Study the drawing (mm; zero at the part's minimum x, y, z) and answer. Round coordinates to 2 decimals unless told otherwise and drop trailing zeros. Loops run counter-clockwise (first coordinate to the right, second up) from the corner with the lowest first, then second, coordinate; pieces in that order, holes last. Notation, with made-up numbers: (43, 50) -> (86, 50) arc R26 cw to (86, 65) -> close; hole circle Ø2 at (77.5, 3.25). An arc over 180 degrees is marked (long way). Answer in a Markdown table with one row per item. Add a question column.
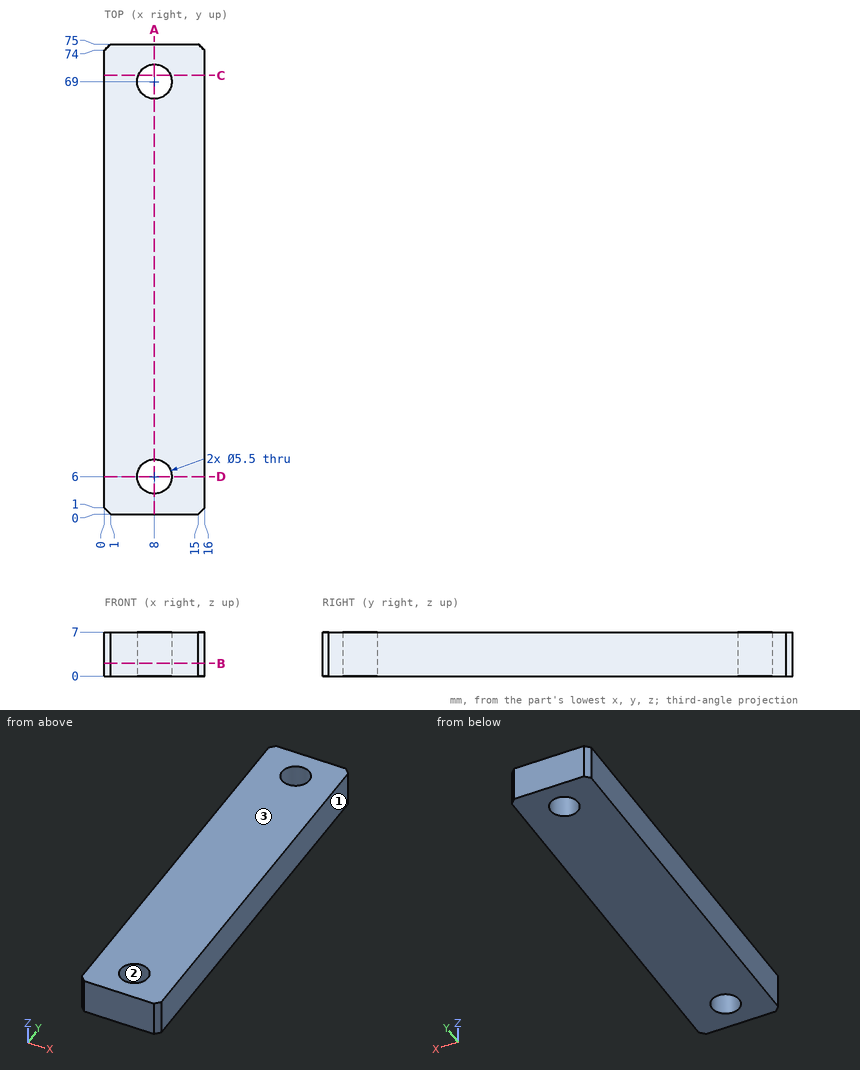
Item 1: Section D-D, the plane y = 6 is taken. Write down the section's boundary in (x, z).
Item 2: Section B-B, the plane z = 2 is taken. Write down the section's boundary in (x, y).
Item 3: Section A-A, the plane x = 8 is taken. Write down the section's boundary in (y, z).
Item 4: The mould has two halves that part along X. Classify the marked faces 1, 2 and 3: +X half, -X half, draft (parallel to the pull), parting line (faces both ways), or undercut.
Item 5: Flat-ended cylindrical pins translate along their axes: P1, Ø6.5, axis at x = 8, y = 6, coming from the +Z side; P2, Ø5, axis at x = 8, y = 69, coming from the +Z side. Find the tip coordinate at first contact, or state that the pin passes through.
Item 6: Section C-C, the plane y = 70 is taken. Write down the section's boundary in (x, z), and give its area (3 significant figures).
Item 7: Consider L1, parallel to Y at x = 8, z = 3.5; L2, parallel to Y at x = 6, z = 2.25; L3, parallel to X at y = 6.5, z = 3. Determine where each line is inside the solid, lowest interval first. Write a range as from..to.
Here are the results:
| question | item | result |
|---|---|---|
| 1 | outline | (0, 0) -> (5.25, 0) -> (5.25, 7) -> (0, 7) -> close; (10.75, 0) -> (16, 0) -> (16, 7) -> (10.75, 7) -> close |
| 2 | outline | (0, 1) -> (1, 0) -> (15, 0) -> (16, 1) -> (16, 74) -> (15, 75) -> (1, 75) -> (0, 74) -> close; hole circle Ø5.5 at (8, 6); hole circle Ø5.5 at (8, 69) |
| 3 | outline | (0, 0) -> (3.25, 0) -> (3.25, 7) -> (0, 7) -> close; (8.75, 0) -> (66.25, 0) -> (66.25, 7) -> (8.75, 7) -> close; (71.75, 0) -> (75, 0) -> (75, 7) -> (71.75, 7) -> close |
| 4 | face 1 | +X half |
| 4 | face 2 | undercut |
| 4 | face 3 | draft |
| 5 | P1 | stops at z = 7 |
| 5 | P2 | passes through |
| 6 | outline | (0, 0) -> (5.44, 0) -> (5.44, 7) -> (0, 7) -> close; (10.56, 0) -> (16, 0) -> (16, 7) -> (10.56, 7) -> close |
| 6 | area | 76.1 mm² |
| 7 | L1 | y = 0..3.25, 8.75..66.25, 71.75..75 |
| 7 | L2 | y = 0..4.11, 7.89..67.11, 70.89..75 |
| 7 | L3 | x = 0..5.3, 10.7..16 |
